Geometry: final body of the model. Coordinates: model frame, mm. A direction names the side the tool comes from. Round coordinates to 2 decimals unless told otherwise and drop trailing zeros. Loops run counter-clockwise (first coordinate to the right, second up) from the corner with the lowest first, then second, coordinate; pieces in that order, holes last. Notation, with made-up numbers: M -23.75,34.5 L -12.75,34.5 A17 ccw -12.75,56.5 Z; hole C 70,-21.75 d10. An arc over 180 degrees is marked long. Answer as a JSON object with one key per item and string values.
from build123d import *

# Parameters (mm, degrees)
FILLET1_R          = 0.5
SKETCH8_W          = 0.25
SKETCH8_H          = 8
CUT_EXTRUDE1_DEPTH = 6
CIRPATTERN1_COUNT  = 3


with BuildPart() as part:
    # Sketch1 → Revolve1 (revolve)
    with BuildSketch(Plane.XY, mode=Mode.PRIVATE) as revolve1_sk:
        with BuildLine():
            Line((-5, 3.1), (-5, -1))
            Line((-5, -1), (-5.25, -1))
            Line((-5.25, -1), (-5.25, -2))
            Line((-5.25, -2), (-4, -2))
            Line((-4, -2), (-4, -12.6))
            Line((-4, -12.6), (-3.5, -12.6))
            Line((-3.5, -12.6), (-3.5, 0))
            Line((-3.5, 0), (-3.125, 0))
            Line((-3.125, 0), (-3.125, 9.4))
            Line((-3.125, 9.4), (-1.25, 9.4))
            Line((-1.25, 9.4), (-1.25, 10.4))
            Line((-1.25, 10.4), (-5, 10.4))
            Line((-5, 10.4), (-5, 6.5))
            add(Edge.make_bspline(
                [(-5, 6.5), (-5.047605665, 6.363384357), (-5.0814919, 6.202637521), (-5.130093219, 5.840342723), (-5.144049999, 5.645135031), (-5.15, 5.440840859)],
                knots=[0, 0, 0, 0, 0.5, 0.5, 1, 1, 1, 1], degree=3))
            Line((-5.15, 5.440840859), (-5, 5.440840859))
            Line((-5, 5.440840859), (-5, 4.297032053))
            add(Edge.make_bspline(
                [(-5, 4.297032053), (-5.05121173, 4.142122175), (-5.086517142, 3.960249608), (-5.134772947, 3.550843087), (-5.146982855, 3.330472207), (-5.15, 3.1)],
                knots=[0, 0, 0, 0, 0.5, 0.5, 1, 1, 1, 1], degree=3))
            Line((-5.15, 3.1), (-5, 3.1))
        make_face()
    revolve(revolve1_sk.sketch.rotate(Axis((0, -30.576267402, 0), (0, 1, 0)), 270), axis=Axis((0, -30.576267402, 0), (0, 1, 0)))

    # Fillet1
    fillet1_edges = [part.edges().sort_by_distance(p)[0] for p in [
        (0, 10.4, 5),
    ]]
    fillet(fillet1_edges, radius=FILLET1_R)

    # Sketch8 → Cut-Extrude1 (cut, symmetric)
    with BuildSketch(Plane.XY):
        with Locations((0, -8.8)):
            Rectangle(SKETCH8_W, SKETCH8_H)
    cut_extrude1 = extrude(amount=CUT_EXTRUDE1_DEPTH, both=True, mode=Mode.SUBTRACT)

    # CirPattern1: Cut-Extrude1 ×3 about axis
    cirpattern1_axis = Axis((0, 0, 0), (0, 1, 0))
    for i in range(1, CIRPATTERN1_COUNT):
        add(cut_extrude1.rotate(cirpattern1_axis, i * 360 / CIRPATTERN1_COUNT), mode=Mode.SUBTRACT)


solid = part.part
1) Ray query, line 1 (X direction, y = 5, z = 0) (3 decimals); line 2 (X direction, y = 9.75, z = 0); line 3 (Y direction, x = 0.5, z = 3.25). Return the intervals inside material, ascending.
Results:
{"line 1": "-5 to -3.125, 3.125 to 5", "line 2": "-5 to -1.25, 1.25 to 5", "line 3": "0 to 10.4"}
2) Pull-direction query (X, two-part tool) for faces 4 (the flat face through (1, 9.4, -1)), 5 (the flat face through (3.7, -12.6, 0)), 6 (the cylindrical face through (-0.94, 4.77, -2.98)), 7 (the cylindrical face through (4.88, 1.02, 1.08)); classes: +X half, -X half, draft (parallel to the pull), parting line (faces both ways), or undercut.
Results:
{"face 4": "undercut", "face 5": "draft", "face 6": "undercut", "face 7": "parting line"}
3) Section query B-B (y = 9). Return the cut outline in (x, z) (3 decimals).
Results:
{"outline": "C 0,0 d10; hole C 0,0 d6.25"}
4) Reachability of faces 1 (the cylindrical face through (3.905, -7.374, 0.867)), 2 (the cylindrical face through (4.88, 8.18, 1.08)), 3 (the flat face through (-3.7, -12.6, 0)) from +Z, -Z, +X, -X, +Y, -Y: full face, straight path, thin tool, end or side. Return the list, or none.
Results:
{"face 1": "-Y", "face 2": "+Y", "face 3": "+Z, -Z, +X, -X, -Y"}
5) Pin query (flat end, axial travel): P1, Ø4, axis at x = 3, y = 5.5, coming from the -Z side; P2, Ø1, axis at x = -2.5, y = 1, coming from the -Z side; P3, Ø3, axis at x = 1.5, y = 5, coming from the +Z side. Return the tip coordinate at first contact, or that it passes through.
Results:
{"P1": "z = -5.05", "P2": "z = -4.58", "P3": "z = 5.15"}
6) Section query A-A (y = -7.5). Return the cut outline in (x, z) (3 decimals).
Results:
{"outline": "M -3.525,-1.891 L -3.092,-1.641 A3.5 cw -3.092,1.641 L -3.525,1.891 A4 ccw Z; M -3.4,-2.107 A4 ccw -0.125,-3.998 L -0.125,-3.498 A3.5 cw -2.967,-1.857 Z; M -3.4,2.107 L -2.967,1.857 A3.5 cw -0.125,3.498 L -0.125,3.998 A4 ccw Z; M 0.125,-3.998 A4 ccw 3.4,-2.107 L 2.967,-1.857 A3.5 cw 0.125,-3.498 Z; M 0.125,3.498 A3.5 cw 2.967,1.857 L 3.4,2.107 A4 ccw 0.125,3.998 Z; M 3.092,-1.641 L 3.525,-1.891 A4 ccw 3.525,1.891 L 3.092,1.641 A3.5 cw Z"}
